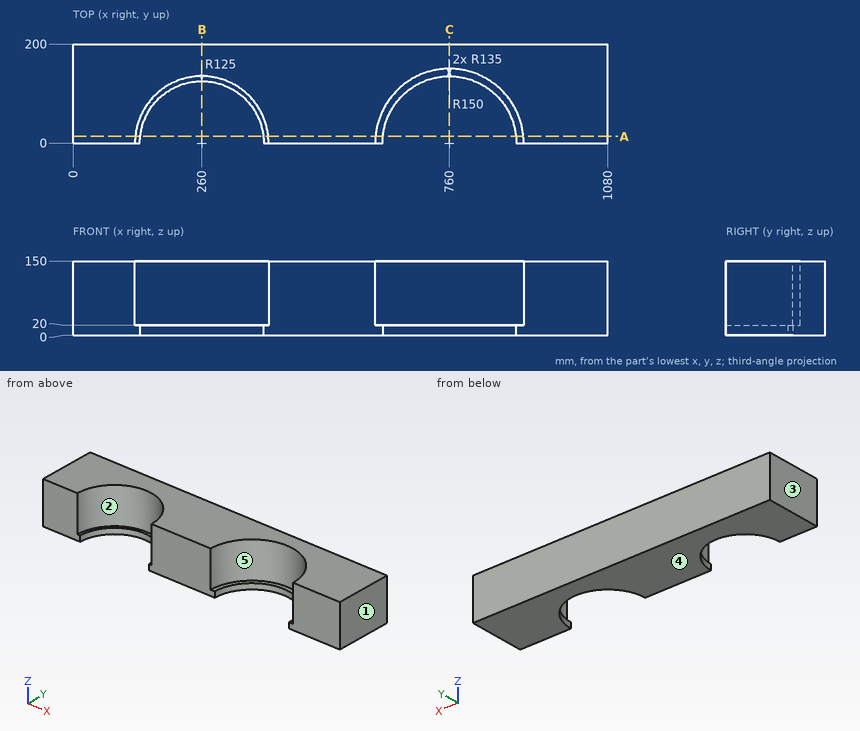
Source: three-view drawing plus pictorial views. Frame: mm from the lowest corner of the part. A direction names the side the tool comes from. Coordinates: 2 decimals unless noted, no trailing zeros. Order: outer loops, then holes, each group sorted by start corner. A loop starts at its lowest first (then second) coordinate and runs counter-clockwise, first axis right, second up. Notation, with made-up numbers: M 84,14 L 142,14 A19 ccw 142,45 Z; hole C 89.5,25.25 d8. An arc over 180 degrees is marked long. Write each question's results on one line, items separated by ' | '. Start each with the question number.
1. Material intervals for L1, parallel to X at y = 62, z = 17; L2, parallel to X at y = 26.5, z = 135; L3, parallel to Z at x = 695, y = 131.5, sorted ascending.
2. Section B-B, the plane x = 260. Return the cut outline in (y, z).
3. Reachability of the marked faces 1 and 2 from +Z, -Z, +X, -X, +Y, -Y: full face, straight path, thin tool, end or side. Return the list, or none.
4. Section A-A, the plane y = 13.5. Return the cut outline in (x, z).
5. Pin query (flat end, axial travel): pin 1 (3 mm diameter, centred on x = 787.5, z = 36.5, fed in from -Y). Return the tip coordinate at first contact, or that it passes through.
6. Draft query along X for the marked faces 3, 4 and 5. Return one class per face: +X half, -X half, draft (parallel to the pull), parting line (faces both ways), or undercut.
7. Section C-C, the plane x = 760. Return the cut outline in (y, z).
Solution:
1) L1: 0 to 151.46, 368.54 to 640.08, 879.92 to 1080 | L2: 0 to 127.63, 392.37 to 612.36, 907.64 to 1080 | L3: 0 to 20
2) outline: M 125,0 L 200,0 L 200,150 L 135,150 L 135,20 L 125,20 Z
3) face 1: +Z, -Z, +X, +Y, -Y | face 2: +Z, -Y
4) outline: M 0,0 L 135.73,0 L 135.73,20 L 125.68,20 L 125.68,150 L 0,150 Z; M 384.27,0 L 625.68,0 L 625.68,20 L 610.61,20 L 610.61,150 L 394.32,150 L 394.32,20 L 384.27,20 Z; M 894.32,0 L 1080,0 L 1080,150 L 909.39,150 L 909.39,20 L 894.32,20 Z
5) pin 1: y = 147.17
6) face 3: -X half | face 4: draft | face 5: undercut
7) outline: M 135,0 L 200,0 L 200,150 L 150,150 L 150,20 L 135,20 Z
